Verification items for the finished model (mm, model axes). A direction names the side the tool comes from. Round coordinates to 2 decimals unless told otherwise and drop trailing zeros. Order: outer loops, then holes, each group sorted by start corner. A loop starts at its lowest first (then second) coordinate and runs counter-clockwise, first axis right, second up. Notation, with made-up numbers: M 84.25,-37.75 L 110.25,-37.75 A16 ccw 110.25,-18.75 Z; hole C 37.5,44.5 d5. An arc over 180 degrees is marked long. Use one line per item in the form item = value. Start each with the question number.
Item 1: Thickness scan on probe 1 along X at (y, z) = (0, -1.75); probe 2 along Y at (x, z) = (30, -7.5); probe 3 along Y at (x, z) = (30, 8). Record the ranges inside material, lowest first. Write a range as [from, to].
Item 2: Tool access check on faces 5 (the flat face through (-26, 4, 0)), 6 (the cylindrical face through (-48, 19, 0)), 7 (the cylindrical face through (56.409, 0.33, 7.493)). Record the directions out of +Z, -Z, +X, -X, +Y, -Y that give a thin tool (end or side, any length) a straight path to the whole face; none if there is none.
Item 3: Cross-section at B-B on y = 1. Count the separate pieces of the cut face and the enclosed holes in it, then the cut area to 3 significant figures.
Item 4: Cross-section at A-A on x = 30. Enter the section's corners in (y, z), then the cut area to 3 significant figures.
Item 5: Go/stop test with a flat-tipped pin: pin 1 Ø2 at (y, z) = (5, -6) entering from +X. Record where the tip stops, or that it passes through.
Item 6: Release check for a two-part mould opening along Y. For faces 1 (the cylindrical face through (49, 18, 0)), 2 (the cylindrical face through (-39, 0, 5)), 3 (the cylindrical face through (24.505, 0.242, -5.07)), 4 (the flat face through (65, 0, 0)) record: +Y half, -Y half, draft (parallel to the pull), parting line (faces both ways), or undercut.
from build123d import *

# Parameters (mm, degrees)
SKETCH1_W           = 100
SKETCH1_H           = 40
SKETCH1_R           = 5.5
BOSS_EXTRUDE1_DEPTH = 10
SKETCH2_R           = 7.5
BOSS_EXTRUDE2_DEPTH = 15
FILLET1_R           = 2
SKETCH3_R           = 9
CUT_EXTRUDE1_DEPTH  = 10
FILLET2_R           = 5


with BuildPart() as part:
    # Sketch1 → Boss-Extrude1 (new, symmetric)
    with BuildSketch(Plane.XY):
        Rectangle(SKETCH1_W, SKETCH1_H)
        with Locations((-30, 0)):
            Circle(SKETCH1_R, mode=Mode.SUBTRACT)
        with Locations((30, 0)):
            Circle(SKETCH1_R, mode=Mode.SUBTRACT)
    extrude(amount=BOSS_EXTRUDE1_DEPTH, both=True)

    # Sketch2 → Boss-Extrude2 (add)
    with BuildSketch(Plane(origin=(50, 0, 0), x_dir=(0, 0, -1), z_dir=(1, 0, 0))):
        Circle(SKETCH2_R)
    extrude(amount=BOSS_EXTRUDE2_DEPTH)

    # Fillet1
    fillet1_edges = [part.edges().sort_by_distance(p)[0] for p in [
        (65, 0, 7.5),
    ]]
    fillet(fillet1_edges, radius=FILLET1_R)

    # Sketch3 → Cut-Extrude1 (cut)
    with BuildSketch(Plane.XY.offset(10)):
        with Locations((-30, 0)):
            Circle(SKETCH3_R)
        with Locations((30, 0)):
            Circle(SKETCH3_R)
    extrude(amount=-CUT_EXTRUDE1_DEPTH, mode=Mode.SUBTRACT)

    # Fillet2
    fillet2_edges = [part.edges().sort_by_distance(p)[0] for p in [
        (50, -20, 0),
        (-50, -20, 0),
        (-50, 20, 0),
        (50, 20, 0),
    ]]
    fillet(fillet2_edges, radius=FILLET2_R)


solid = part.part
Output values:
q1.probe_1 = [-50, -35.5], [-24.5, 24.5], [35.5, 65]
q1.probe_2 = [-20, -5.5], [5.5, 20]
q1.probe_3 = [-20, -9], [9, 20]
q2.face_5 = +Z
q2.face_6 = +Z, -Z, -X, +Y
q2.face_7 = +X
q3.separate_pieces = 3
q3.enclosed_holes = 0
q3.area = 1,650 mm2
q4.outline = M -20,-10 L -5.5,-10 L -5.5,0 L -9,0 L -9,10 L -20,10 Z; M 5.5,-10 L 20,-10 L 20,10 L 9,10 L 9,0 L 5.5,0 Z
q4.area = 510 mm2
q5.pin_1 = 64.51
q6.face_1 = +Y half
q6.face_2 = undercut
q6.face_3 = undercut
q6.face_4 = draft
